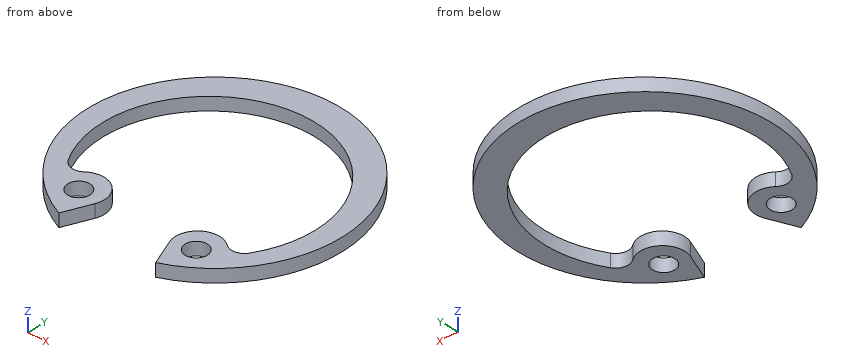
```python
from build123d import *

# Parameters (mm, degrees)
SKETCH_1_R        = 0.85
EXTRUDE_967_DEPTH = 1


with BuildPart() as part:
    # 草图1 → Extrude 967 (new body)
    with BuildSketch(Plane.XY):
        with BuildLine():
            Line((-2.870026243, -6.928856281), (-3.731163466, -9.007825442))
            ThreePointArc((-3.731163466, -9.007825442), (0, 9.75), (3.731163466, -9.007825442))
            Line((3.731163466, -9.007825442), (2.870026243, -6.928856281))
            ThreePointArc((2.870026243, -6.928856281), (3.421390109, -4.91771829), (5.506424922, -4.953884028))
            ThreePointArc((5.506424922, -4.953884028), (6.309138908, -5.1592502), (6.991181868, -4.688779786))
            ThreePointArc((6.991181868, -4.688779786), (0, 7.65), (-6.991181868, -4.688779786))
            ThreePointArc((-6.991181868, -4.688779786), (-6.309138908, -5.1592502), (-5.506424922, -4.953884028))
            ThreePointArc((-5.506424922, -4.953884028), (-3.421390109, -4.91771829), (-2.870026243, -6.928856281))
        make_face()
        with Locations((-4.522967504, -6.47709541)):
            Circle(SKETCH_1_R, mode=Mode.SUBTRACT)
        with Locations(Location((4.522967504, -6.47709541, 0), (0, 0, 180))):
            Circle(SKETCH_1_R, mode=Mode.SUBTRACT)
    extrude(amount=EXTRUDE_967_DEPTH)


solid = part.part
```
The listing builds one solid part. Answer for the finished solid, in the listing's coordinates (mm). Round coordinates to 2 decimals unless told otherwise and drop trailing zeros. Loops run counter-clockwise (first coordinate to the right, second up) from the corner with the lowest first, then second, coordinate; pieces in that order, holes last.
Q1. Section D-D, the plane x = 0 is taken. Determine the outline of the cut face in (y, z).
Q2. Section B-B, the plane x = -6 is taken. Determine the outline of the cut face in (y, z), then the cut area to 3 significant figures.
Q3. Find the intervals of material crossed by line 1 (X direction, y = -6, z = 0.6); line 2 (Y direction, x = 5, z = 0.7); line 3 (X direction, y = -6.5, z = 0.8), in increasing order.
Q4. Section C-C, the plane z = 0.3 is taken. Determine the outline of the cut face in (x, y), then the cut area to 3 significant figures.
Q5. Given pin 1 Ø10 at (x, y) = (-6, 3) entering from -Z, flat-ended and moving along its own axis, determine where the tip first touches the part or whether it passes through.
Q6. Section A-A, the plane y = 2.25 is taken. Determine the outline of the cut face in (x, z).
Completed:
1. outline: (7.65, 0) - (9.75, 0) - (9.75, 1) - (7.65, 1) - close
2. outline: (-7.69, 0) - (-5.17, 0) - (-5.17, 1) - (-7.69, 1) - close; (5.02, 0) - (7.69, 0) - (7.69, 1) - (5.02, 1) - close
2. area: 5.19 mm2
3. line 1: x = -7.69 to -5.23, -3.82 to -2.76, 2.76 to 3.82, 5.23 to 7.69
3. line 2: y = -8.37 to -7.18, -5.77 to -4.67, 5.94 to 8.37
3. line 3: x = -7.27 to -5.37, -3.67 to -2.76, 2.76 to 3.67, 5.37 to 7.27
4. outline: (-6.99, -4.69) arc R8.15 cw (long way) to (6.99, -4.69) arc R1 cw to (5.51, -4.95) arc R1.7 ccw to (2.87, -6.93) - (3.73, -9.01) arc R9.75 ccw (long way) to (-3.73, -9.01) - (-2.87, -6.93) arc R1.7 ccw to (-5.51, -4.95) arc R1 cw to start; hole circle Ø1.7 at (-4.52, -6.48); hole circle Ø1.7 at (4.52, -6.48)
4. area: 92.9 mm2
5. pin 1: stops at z = 0
6. outline: (-9.49, 0) - (-7.67, 0) - (-7.67, 1) - (-9.49, 1) - close; (7.67, 0) - (9.49, 0) - (9.49, 1) - (7.67, 1) - close
